Source: CAD feature listing. Evaluate the final solid. Frame: model axes, mm. Round coordinates to 2 decimals unless told otherwise and drop trailing zeros. Write each loop counter-clockwise with the first axis right and the second up, starting at its lowest first coordinate (ties: lowest second). Pieces come first, ordered by that corner, then holes. Notation, with made-up numbers: (-4, 2) -> (18, 2) arc R31 cw to (18, 38) -> close; hole circle Ø10 at (-28.75, 68.25). An arc over 180 degrees is marked (long way). Return JSON: item names as keys, results as strings. Group by question number.
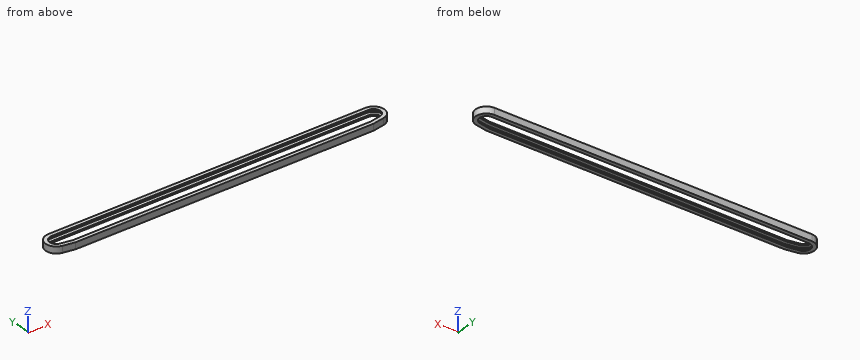
from build123d import *

# Parameters (mm, degrees)
BOSS_EXTRUDE1_DEPTH = 10
CUT_EXTRUDE1_DEPTH  = 5


with BuildPart() as part:
    # Sketch2 → Boss-Extrude1 (new, symmetric)
    with BuildSketch(Plane.XY):
        with BuildLine():
            Line((-485, 32.5), (485, 32.5))
            ThreePointArc((485, 32.5), (517.376327688, 2.832561639), (490.643565774, -32.006251973))
            Line((490.643565774, -32.006251973), (455.524931981, -38.198614636))
            Line((455.524931981, -38.198614636), (-455.524931981, -38.198614636))
            Line((-455.524931981, -38.198614636), (-490.643565774, -32.006251973))
            ThreePointArc((-490.643565774, -32.006251973), (-517.376327688, 2.832561639), (-485, 32.5))
        make_face()
        with BuildLine():
            Line((-485, 20.5), (485, 20.5))
            ThreePointArc((485, 20.5), (505.421991311, 1.786692726), (488.559787642, -20.188558937))
            Line((488.559787642, -20.188558937), (454.475068019, -26.198614636))
            Line((454.475068019, -26.198614636), (-454.475068019, -26.198614636))
            Line((-454.475068019, -26.198614636), (-488.559787642, -20.188558937))
            ThreePointArc((-488.559787642, -20.188558937), (-505.421991311, 1.786692726), (-485, 20.5))
        make_face(mode=Mode.SUBTRACT)
    extrude(amount=BOSS_EXTRUDE1_DEPTH, both=True)

    # Sketch8 → Cut-Extrude1 (cut, symmetric)
    with BuildSketch(Plane.XY):
        with BuildLine():
            Line((455.437443318, -37.198614636), (490.469917597, -31.02144422))
            ThreePointArc((490.469917597, -31.02144422), (516.38013299, 2.745405897), (485, 31.5))
            Line((485, 31.5), (-485, 31.5))
            ThreePointArc((-485, 31.5), (-516.38013299, 2.745405897), (-490.469917597, -31.02144422))
            Line((-490.469917597, -31.02144422), (-455.437443318, -37.198614636))
            Line((-455.437443318, -37.198614636), (455.437443318, -37.198614636))
        make_face()
    extrude(amount=CUT_EXTRUDE1_DEPTH, both=True, mode=Mode.SUBTRACT)


solid = part.part
Item 1: Cut plane A-A on x = 382. Output: boundary loops of the cut face in (y, z).
Item 2: First-contact query: pin 1 Ø8 at (y, z) = (9, -7) entering from -X; pin 2 Ø2 at (y, z) = (7, 0.5) entering from -X; pin 3 Ø1.5 at (y, z) = (-11.5, 6) entering from +X. Flat tips, straight axial feed; report the tip coordinate or a pass-through.
Item 3: Cut plane B-B on z = -1. Output: boundary loops of the cut face in (x, y).
Item 4: Cut plane C-C on y = -6. Output: boundary loops of the cut face in (x, z).
Item 5: Material intervals for probe 1 along Z at (x, y) = (176.5, -30); probe 2 along Y at (x, z) = (300.5, 5.25); probe 3 along Y at (x, z) = (-165, -3), sorted ascending.
Here are the results:
{
 "1": {"outline": "(-38.2, -10) -> (-26.2, -10) -> (-26.2, -5) -> (-37.2, -5) -> (-37.2, 5) -> (-26.2, 5) -> (-26.2, 10) -> (-38.2, 10) -> close; (20.5, -10) -> (32.5, -10) -> (32.5, 10) -> (20.5, 10) -> (20.5, 5) -> (31.5, 5) -> (31.5, -5) -> (20.5, -5) -> close"},
 "2": {"pin 1": "stops at x = -517.11", "pin 2": "stops at x = -516.94", "pin 3": "stops at x = 515.67"},
 "3": {"outline": "(-490.64, -32.01) -> (-455.52, -38.2) -> (455.52, -38.2) -> (490.64, -32.01) arc R32.5 ccw to (485, 32.5) -> (-485, 32.5) arc R32.5 ccw to start; hole (-490.47, -31.02) -> (-455.44, -37.2) -> (455.44, -37.2) -> (490.47, -31.02) arc R31.5 ccw to (485, 31.5) -> (-485, 31.5) arc R31.5 ccw to start"},
 "4": {"outline": "(-516.94, -10) -> (-504.6, -10) -> (-504.6, -5) -> (-515.92, -5) -> (-515.92, 5) -> (-504.6, 5) -> (-504.6, 10) -> (-516.94, 10) -> close; (504.6, -10) -> (516.94, -10) -> (516.94, 10) -> (504.6, 10) -> (504.6, 5) -> (515.92, 5) -> (515.92, -5) -> (504.6, -5) -> close"},
 "5": {"probe 1": "z = -10 to -5, 5 to 10", "probe 2": "y = -38.2 to -26.2, 20.5 to 32.5", "probe 3": "y = -38.2 to -37.2, 31.5 to 32.5"}
}
